Verification items for the finished model (mm, model axes). Coordinates: 2 decimals unless noted, no trailing zeros. Write each loop counter-clockwise with the first axis right and the second up, starting at its lowest first coordinate (ties: lowest second). Pieces come first, ordered by that corner, then holes. Notation, with made-up numbers: M 40.25,-15.75 L 77.25,-15.75 A25 ccw 77.25,-1.75 Z; hole C 51,22 d9. An arc over 180 degrees is marked long. Answer in a Markdown table with one row per item.
from build123d import *

# Parameters (mm, degrees)
BOSS_EXTRUDE1_DEPTH = 10
CHAMFER1_SIZE       = 0.5


with BuildPart() as part:
    # Sketch1 → Boss-Extrude1 (new body)
    with BuildSketch(Plane.XY):
        with BuildLine():
            Line((0, 6), (60, 6))
            ThreePointArc((60, 6), (66, 0), (60, -6))
            Line((60, -6), (0, -6))
            ThreePointArc((0, -6), (-6, 0), (0, 6))
        make_face()
    extrude(amount=BOSS_EXTRUDE1_DEPTH)

    # Chamfer1
    chamfer1_edges = [part.edges().sort_by_distance(p)[0] for p in [
        (66, 0, 10),
        (30, 6, 10),
        (-6, 0, 10),
        (30, 6, 0),
        (66, 0, 0),
        (30, -6, 0),
        (-6, 0, 0),
        (30, -6, 10),
    ]]
    chamfer(chamfer1_edges, length=CHAMFER1_SIZE)


solid = part.part
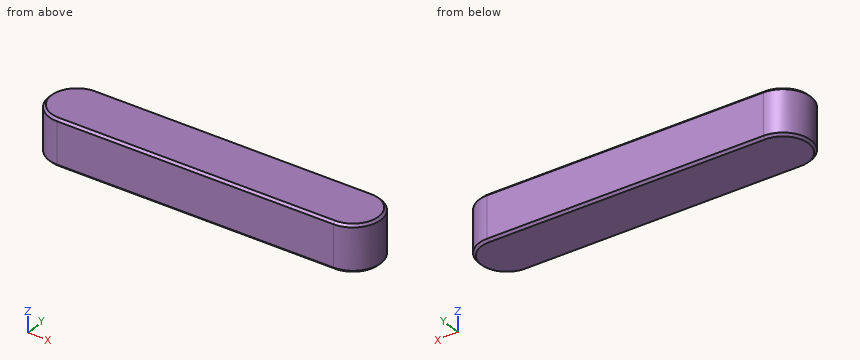
1) Sectioned sample at A-A (z = 7.5). Record the cut outline in (x, y).
Response values:
| item | result |
|---|---|
| outline | M 0,-6 L 60,-6 A6 ccw 60,6 L 0,6 A6 ccw Z |
2) Thickness scan on L1, parallel to X at y = -3.75, z = 2; L2, parallel to X at y = 2, z = 8.75; L3, parallel to Y at x = -2.5, z = 4.75. Record the ranges inside material, lowest first. Write a range as [from, to].
Response values:
| item | result |
|---|---|
| L1 | x = [-4.68, 64.68] |
| L2 | x = [-5.66, 65.66] |
| L3 | y = [-5.45, 5.45] |
3) Depth check by flat-ended pin: pin 1 (1 mm diameter, centred on y = -0.5, z = 6, fed in from -X); pin 2 (1 mm diameter, centred on y = 3, z = 8.5, fed in from +X). Enter the tip coordinate at first touch or a pass-through.
Response values:
| item | result |
|---|---|
| pin 1 | stops at x = -6 |
| pin 2 | stops at x = 65.45 |
